Verification items for this drawing (mm, ordinates from the low corner). Coordinates: 2 decimals unless noted, no trailing zeros. Loops run counter-clockwise (first coordinate to the right, second up) from the corner with the lowest first, then second, coordinate; pieces in that order, holes last. Notation, with made-up numbers: (71, 3.5) - (118, 3.5) arc R9 cw to (118, 20.5) - close; hole circle Ø9 at (41, 31.25). An arc over 180 degrees is marked (long way). Write each question's results on one line, items separated by ' | '. Start each with the question number.
(1) Sectioned sample at A-A (y = 335). Enter the section's corners in (x, z), plus the area to 3 significant figures.
(2) Sectioned sample at C-C (y = 253.5). Enter the section's corners in (x, z), plus the area to 3 significant figures.
(3) Material ranges on probe 1 along Y at (x, z) = (670, 18); probe 2 along X at (y, z) = (249, 6.25); probe 3 along Y at (x, z) = (333, 3), recorded low to high.
(4) Sectioned sample at B-B (x = 50). Enter the section's corners in (y, z), plus the area to 4 significant figures.
(5) Go/stop test with a flat-tipped pin: pin 1 Ø3 at (x, z) = (481, 4) entering from +Y. Record where the tip stops, or that it passes through.
(6) Sectioned sample at D-D (z = 18). Enter the section's corners in (x, y), plus the area to 3 significant figures.
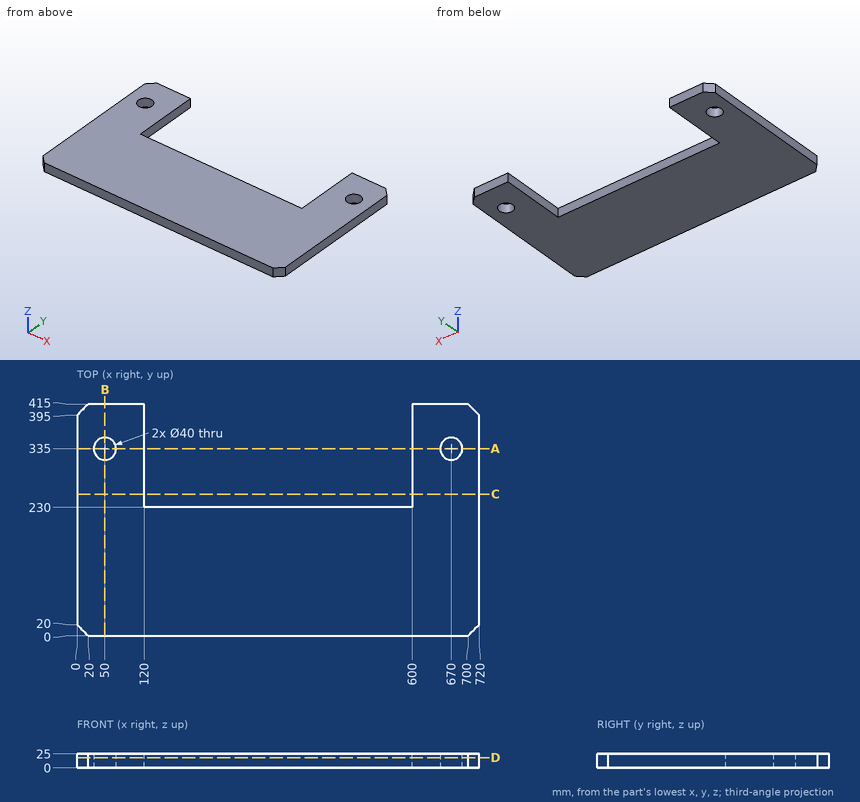
Outcome:
1) outline: (0, 0) - (30, 0) - (30, 25) - (0, 25) - close; (70, 0) - (120, 0) - (120, 25) - (70, 25) - close; (600, 0) - (650, 0) - (650, 25) - (600, 25) - close; (690, 0) - (720, 0) - (720, 25) - (690, 25) - close | area: 4,000 mm2
2) outline: (0, 0) - (120, 0) - (120, 25) - (0, 25) - close; (600, 0) - (720, 0) - (720, 25) - (600, 25) - close | area: 6,000 mm2
3) probe 1: y = 0 to 315, 355 to 415 | probe 2: x = 0 to 120, 600 to 720 | probe 3: y = 0 to 230
4) outline: (0, 0) - (315, 0) - (315, 25) - (0, 25) - close; (355, 0) - (415, 0) - (415, 25) - (355, 25) - close | area: 9,375 mm2
5) pin 1: stops at y = 230
6) outline: (0, 20) - (20, 0) - (700, 0) - (720, 20) - (720, 395) - (700, 415) - (600, 415) - (600, 230) - (120, 230) - (120, 415) - (20, 415) - (0, 395) - close; hole circle Ø40 at (50, 335); hole circle Ø40 at (670, 335) | area: 207,000 mm2
